Input: part model. Units: mm. Frame: model coordinates. Face numbers are marked on the shaded views. A direction names the side the tool comes from. Round coordinates to 2 decimals unless told otherwise and drop trailing zeros. Write each loop counter-clockwise with the first axis right and the second up, starting at its lowest first coordinate (ties: lowest second). Pieces come first, ordered by that corner, then holes. Notation, with made-up numbers: (37, -36.5) -> (46, -36.5) arc R18 ccw to (46, -6.5) -> close; hole circle Ø8 at (39, 38.25). An arc over 180 degrees is marked (long way). Use CSV: the item, a comma, the result in double quotes.
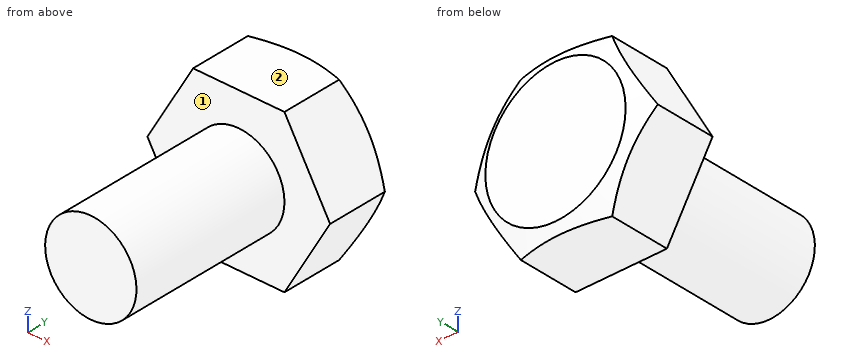
```python
from build123d import *

# Parameters (mm, degrees)
BOSS_EXTRUDE1_DEPTH = 4
SKETCH2_OUTSIDE_W   = 45.006
SKETCH2_OUTSIDE_H   = 43.666
SKETCH2_OUTSIDE_R   = 3.838579207
CUT_EXTRUDE1_DEPTH  = 8.729812417
CUT_EXTRUDE1_DRAFT  = -60
SKETCH3_R           = 2.5
BOSS_EXTRUDE2_DEPTH = 9


with BuildPart() as part:
    # Sketch1 → Boss-Extrude1 (new body)
    with BuildSketch(Plane(origin=(0, 0, 0), x_dir=(1, 0, 0), z_dir=(0, 1, 0))):
        Polygon((5, 0), (2.5, 4.330127019), (-2.5, 4.330127019), (-5, 0), (-2.5, -4.330127019), (2.5, -4.330127019), align=None)
    extrude(amount=BOSS_EXTRUDE1_DEPTH)


with BuildPart() as cut_extrude1_tool:
    # Sketch2 outside → Cut-Extrude1 (with draft: the straight prism first)
    with BuildSketch(Plane(origin=(0, 4, 0), x_dir=(1, 0, 0), z_dir=(0, 1, 0))):
        Rectangle(SKETCH2_OUTSIDE_W, SKETCH2_OUTSIDE_H)
        Circle(SKETCH2_OUTSIDE_R, mode=Mode.SUBTRACT)
    extrude(amount=-CUT_EXTRUDE1_DEPTH)
    # Cut-Extrude1: the draft: its side faces are tilted about the plane it starts from
    cut_extrude1_sides = [cut_extrude1_tool.faces().sort_by_distance(p)[0] for p in [
        (0, -0.364906208, 21.833),
        (22.503, -0.364906208, 0),
        (0, -0.364906208, -21.833),
        (-22.503, -0.364906208, 0),
        (-3.838579207, -0.364906208, 0),
    ]]
    draft(cut_extrude1_sides, Plane(origin=(0, 4, 0), x_dir=(1, 0, 0), z_dir=(0, 1, 0)), CUT_EXTRUDE1_DRAFT)


with BuildPart() as part_1:
    add(part.part)

    # Cut-Extrude1: cut by cut_extrude1_tool
    add(cut_extrude1_tool.part, mode=Mode.SUBTRACT)

    # Sketch3 → Boss-Extrude2 (add)
    with BuildSketch(Plane.XZ):
        with Locations(Location((0, 0, 0), (0, 0, 90))):
            Circle(SKETCH3_R)
    extrude(amount=BOSS_EXTRUDE2_DEPTH)


solid = part_1.part
```
Item 1: Section query C-C on y = -6.5. Return the cut outline in (x, z).
Worked answers:
outline,"circle Ø5 at (0, 0)"
Item 2: First-contact query: pin 1 Ø3 at (x, y) = (-3.5, -4.5) entering from -Z; pin 2 Ø3 at (y, z) = (-3.5, 1.5) entering from +X; pin 3 Ø6 at (x, y) = (-2.5, -7.5) entering from +Z. Flat tips, straight axial feed; report the tip coordinate or a pass-through.
Worked answers:
pin 1,"stops at z = -1.5"
pin 2,"stops at x = 2.5"
pin 3,"stops at z = 2.5"
Item 3: Section query B-B on x = 0. Return the cut outline in (y, z).
Worked answers:
outline,"(-9, -2.5) -> (0, -2.5) -> (0, -4.33) -> (3.72, -4.33) -> (4, -3.84) -> (4, 3.84) -> (3.72, 4.33) -> (0, 4.33) -> (0, 2.5) -> (-9, 2.5) -> close"
Item 4: Section query A-A on y = 1.5. Return the cut outline in (x, z), plus the area to 3 significant figures.
Worked answers:
outline,"(-5, 0) -> (-2.5, -4.33) -> (2.5, -4.33) -> (5, 0) -> (2.5, 4.33) -> (-2.5, 4.33) -> close"
area,"65.0 mm²"
Item 5: Set-up query: the marked faces 1 and 2. Return all of +Z, -Z, +X, -X, +Y, -Y with unobstructed straight access to the full face (end or side cutting, diameter ignored); none if empty.
Worked answers:
face 1,"-Y"
face 2,"+Z, +X, -X, +Y, -Y"
Item 6: Line query: line 1 (Y direction, x = 3.5, z = -0.5); line 2 (Y direction, x = 4, z = -1); line 3 (X direction, y = -1.25, z = 1.75). Output: solid intervals per line, ascending.
Worked answers:
line 1,"y = 0 to 4"
line 2,"y = 0 to 3.84"
line 3,"x = -1.79 to 1.79"
